Verification items for this drawing (mm, ordinates from the low corner). A direction names the side the tool comes from. Give positions to 0.01 mm unless a question says otherwise; leave off trailing zeros. Order: outer loops, then holes, each group sorted by start corner. A loop starts at its lowest first (then second) coordinate and runs counter-clockwise, first axis right, second up.
(1) Sectioned sample at C-C on z = 45.5. Record the cut outline in (x, y), plus the area to 3 significant figures.
(2) Gauge pin test, flat ends, axial feed: pin 1 (15.5 mm diameter, centred on y = 26.5, z = 27, fed in from -X); pin 2 (6 mm diameter, centred on x = 15, z = 30.5, fed in from -Y); pin 3 (2 mm diameter, centred on x = 96.5, z = 36.5, fed in from -Y). Record the tip position at first contact, or that the pin passes through.
(3) Sectioned sample at B-B on x = 25. Record the cut outline in (y, z), plus the area to 3 significant figures.
(4) Scan lines: L1, parallel to Z at x = 25, y = 60.75; L2, parallel to Y at x = 24, z = 54.5; L3, parallel to X at y = 52, z = 28. Record each from-to range of solid material in increasing order.
(5) Sectioned sample at A-A on z = 30. Record the cut outline in (x, y), plus the area to 3 significant figures.
(6) Access from +Z, -Z, +X, -X, +Y, -Y to the whole of each face (thin tool, end or side, straight path). Record for the marked faces 1 and 2.
(7) Sectioned sample at D-D on y = 8.5. Record the cut outline in (x, z).
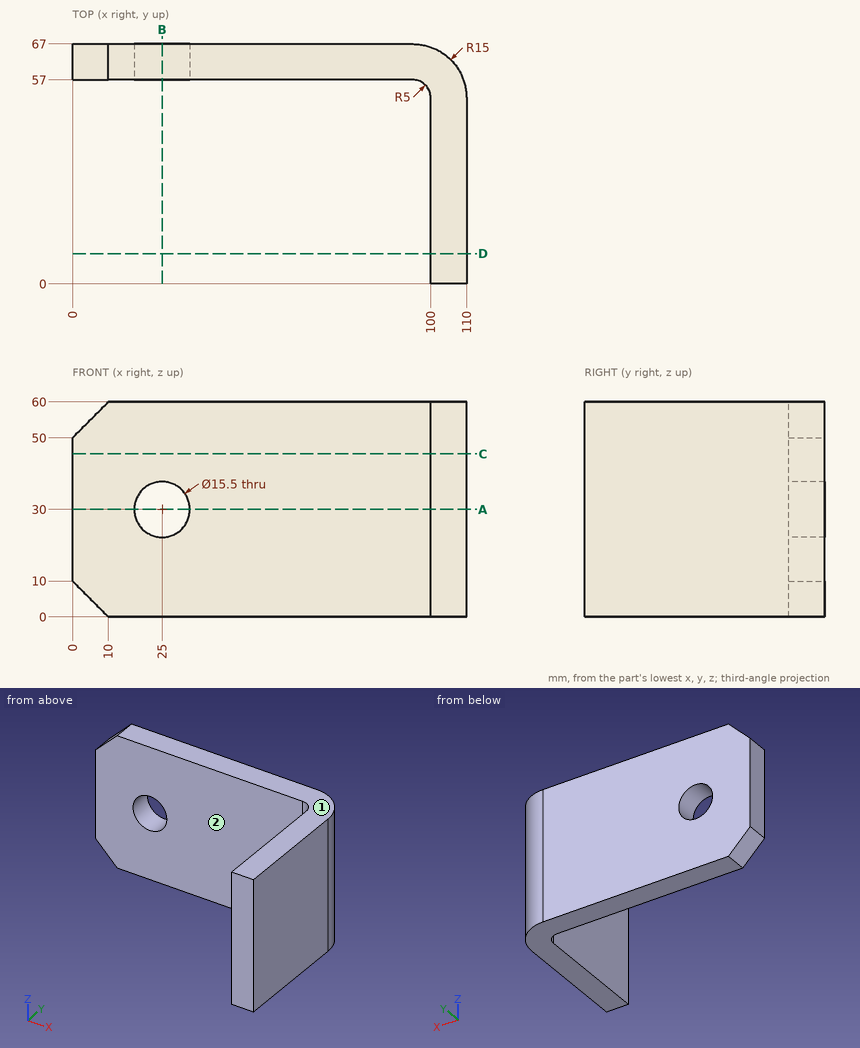
Ans:
1. outline: (0, 57) - (95, 57) arc R5 cw to (100, 52) - (100, 0) - (110, 0) - (110, 52) arc R15 ccw to (95, 67) - (0, 67) - close
1. area: 1,630 mm2
2. pin 1: stops at x = 100
2. pin 2: stops at y = 57
2. pin 3: stops at y = 56.33
3. outline: (57, 0) - (67, 0) - (67, 22.25) - (57, 22.25) - close; (57, 37.75) - (67, 37.75) - (67, 60) - (57, 60) - close
3. area: 445 mm2
4. L1: z = 0 to 22.25, 37.75 to 60
4. L2: y = 57 to 67
4. L3: x = 100 to 110
5. outline: (0, 57) - (17.25, 57) - (17.25, 67) - (0, 67) - close; (32.75, 57) - (95, 57) arc R5 cw to (100, 52) - (100, 0) - (110, 0) - (110, 52) arc R15 ccw to (95, 67) - (32.75, 67) - close
5. area: 1,470 mm2
6. face 1: +Z, +X, -X, +Y, -Y
6. face 2: +Z, -Z, -X, -Y
7. outline: (100, 0) - (110, 0) - (110, 60) - (100, 60) - close
